```python
from build123d import *

# Parameters (mm, degrees)
SKETCH_2_R               = 6.25
CUT_EXTRUDE_1_DEPTH      = 127.688594593
PATTERN_CIRCULAR_1_COUNT = 6
SKETCH_3_R               = 25
CUT_EXTRUDE_2_DEPTH      = 127.688594593
CUT_EXTRUDE_START        = -15
CUT_EXTRUDE_3_DEPTH      = 15
PATTERN_CIRCULAR_2_COUNT = 6
PATTERN_CIRCULAR_3_COUNT = 6


with BuildPart() as part:
    # 草图1 → 旋转1 (revolve)
    with BuildSketch(Plane.XY, mode=Mode.PRIVATE) as revolve_1_sk:
        Polygon((0, 0), (0, 85), (30, 85), (30, 45), (40, 45), (40, 30), (30, 30), (30, 0), align=None)
    revolve(revolve_1_sk.sketch.rotate(Axis((0, 0, 0), (1, 0, 0)), 90), axis=Axis((0, 0, 0), (1, 0, 0)))

    # 草图2 → 切除-拉伸1 (cut, through all)
    with BuildSketch(Plane.ZY):
        with Locations((0, 70)):
            Circle(SKETCH_2_R)
    cut_extrude_1 = extrude(amount=-CUT_EXTRUDE_1_DEPTH, mode=Mode.SUBTRACT)

    # 阵列(圆周)1: 切除-拉伸1 ×6 about axis
    pattern_circular_1_axis = Axis((0, 0, 0), (1, 0, 0))
    for i in range(1, PATTERN_CIRCULAR_1_COUNT):
        add(cut_extrude_1.rotate(pattern_circular_1_axis, i * 360 / PATTERN_CIRCULAR_1_COUNT), mode=Mode.SUBTRACT)

    # 草图3 → 切除-拉伸2 (cut, through all)
    with BuildSketch(Plane.ZY):
        Circle(SKETCH_3_R)
    extrude(amount=-CUT_EXTRUDE_2_DEPTH, mode=Mode.SUBTRACT)

    # 草图6 → 切除-拉伸3 (cut)
    with BuildSketch(Plane.ZY.offset(CUT_EXTRUDE_START)):
        with BuildLine():
            Line((-16, 70), (-16, 83.480536654))
            ThreePointArc((-16, 83.480536654), (0, 85), (16, 83.480536654))
            Line((16, 83.480536654), (16, 70))
            ThreePointArc((16, 70), (0, 54), (-16, 70))
        make_face()
    cut_extrude_3 = extrude(amount=CUT_EXTRUDE_3_DEPTH, mode=Mode.SUBTRACT)

    # 阵列(圆周)2: 切除-拉伸3 ×6 about axis
    pattern_circular_2_axis = Axis((0, 0, 0), (1, 0, 0))
    for i in range(1, PATTERN_CIRCULAR_2_COUNT):
        add(cut_extrude_3.rotate(pattern_circular_2_axis, i * 360 / PATTERN_CIRCULAR_2_COUNT), mode=Mode.SUBTRACT)

    # 草图8 → M12 螺纹孔1 (revolve, cut)
    with BuildSketch(Plane(origin=(0, 60.621778265, 35), x_dir=(0, 0, 1), z_dir=(0, 1, 0))):
        Polygon((0, 0), (0, 21.064389157), (5.1, 18), (5.1, 0), align=None)
    hole_wizard_m12_1 = revolve(axis=Axis((-6.35, 60.621778265, 35), (1, 0, 0)), mode=Mode.SUBTRACT)

    # 阵列(圆周)3: M12 螺纹孔1 ×6 about axis
    pattern_circular_3_axis = Axis((0, 0, 0), (1, 0, 0))
    for i in range(1, PATTERN_CIRCULAR_3_COUNT):
        add(hole_wizard_m12_1.rotate(pattern_circular_3_axis, i * 360 / PATTERN_CIRCULAR_3_COUNT), mode=Mode.SUBTRACT)


solid = part.part
```
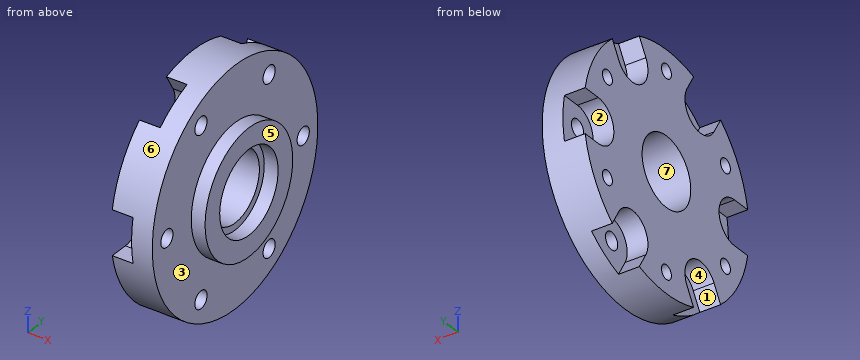
Can you work these out from the model? Positions are in its coordinate system, mm. Face numbers are marked on the shaded views. A direction names the side the tool comes from. Give positions to 0.01 mm unless a question says otherwise; leave off trailing zeros. Write each loop counter-clockwise with the first axis right and the second up, starting at its lowest first coordinate (ties: lowest second). Pieces come first, ordered by that corner, then holes. Notation, with made-up numbers: (10.25, -1) -> (38.25, -1) arc R19 ccw to (38.25, 18) -> close; hole circle Ø2 at (6, 42). An arc over 180 degrees is marked (long way). One line per item, written item: value.
Q1. Imagine slicing it at A-A on z = 0. Please give me the cut outline in (x, y).
Results found:
outline: (0, -54) -> (15, -54) -> (15, -63.75) -> (30, -63.75) -> (30, -45) -> (40, -45) -> (40, -30) -> (30, -30) -> (30, -25) -> (0, -25) -> close; (0, 25) -> (30, 25) -> (30, 30) -> (40, 30) -> (40, 45) -> (30, 45) -> (30, 63.75) -> (15, 63.75) -> (15, 54) -> (0, 54) -> close; (15, -85) -> (30, -85) -> (30, -76.25) -> (15, -76.25) -> close; (15, 76.25) -> (30, 76.25) -> (30, 85) -> (15, 85) -> close
Q2. We'd pull the mould along Z, two halves only. Please class the marked faces 5, 6 and 7: +Z half, -Z half, draft (parallel to the pull), parting line (faces both ways), or undercut.
Results found:
face 5: draft
face 6: parting line
face 7: undercut
Q3. Imagine slicing it at D-D on y = -35. Please give me the cut outline in (x, z).
Results found:
outline: (0, -44.62) -> (15, -44.62) -> (15, -54.37) -> (30, -54.37) -> (30, -28.28) -> (40, -28.28) -> (40, 28.28) -> (30, 28.28) -> (30, 54.37) -> (15, 54.37) -> (15, 44.62) -> (0, 44.62) -> close; (15, -77.46) -> (30, -77.46) -> (30, -66.87) -> (15, -66.87) -> close; (15, 66.87) -> (30, 66.87) -> (30, 77.46) -> (15, 77.46) -> close
Q4. Please list where these lines run through material, in increasing order: line 1 (Y direction, x = 17.5, z = -61); line 2 (Y direction, x = 13.5, z = 35.5); line 3 (Z direction, x = 19, y = 30.5). Write a range as [from, to].
Results found:
line 1: y = [-59.19, -41.24], [-28.76, 28.76], [41.24, 59.19]
line 2: y = [-77.23, -65.7], [-55.55, 55.55], [65.7, 77.23]
line 3: z = [-79.34, -64.96], [-56.28, 56.28], [64.96, 79.34]
Q5. For P1, Ø16.5, axis at y = 0, z = 70, coming from the +X side; P2, Ø6.5, axis at x = 8, y = -77.5, coming from the -Z side; P3, Ø10.5, axis at y = 39.5, z = -55, coming from the -X side, each with a flat end and sliding along its axis, tell me the tip position at first contact or that it passes through.
Results found:
P1: stops at x = 30
P2: stops at z = -41.38
P3: stops at x = 15
Q6. Which directions (+Z, -Z, +X, -X, +Y, -Y) give clear straight access to the entire face, cutting with the end or side of a thin tool? Please do the marked faces 1, 2, 3 and 4.
Results found:
face 1: -Z, -X
face 2: -X, +Y
face 3: +X
face 4: -X
Q7. Imagine slicing it at B-B on y = 73. Please give me the cut outline in (x, z), and give its area (3 significant figures).
Results found:
outline: (0, -43.54) -> (30, -43.54) -> (30, -5.48) -> (15, -5.48) -> (15, -16) -> (0, -16) -> close; (0, 16) -> (15, 16) -> (15, 5.48) -> (30, 5.48) -> (30, 43.54) -> (0, 43.54) -> close
area: 1,970 mm^2
Q8. Imagine slicing it at C-C on x = 27. Please give me the cut outline in (y, z).
Results found:
outline: circle Ø170 at (0, 0); hole circle Ø12.5 at (-70, 0); hole circle Ø12.5 at (-35, -60.62); hole circle Ø12.5 at (-35, 60.62); hole circle Ø50 at (0, 0); hole circle Ø12.5 at (35, -60.62); hole circle Ø12.5 at (35, 60.62); hole circle Ø12.5 at (70, 0)
